Can you work these out from the model? Positions are in its coordinate system, mm. Give positions to 0.01 mm unless a question says otherwise; leave off trailing zeros. Loops run counter-clockwise (first coordinate to the right, second up) from the corner with the lowest first, then second, coordinate; pieces in that order, holes last. Notation, with made-up numbers: (-37.75, -18) - (-25.75, -18) arc R23 ccw to (-25.75, 18) - close; hole circle Ø3 at (-8, -30). An arc over 180 degrees is marked (long way). Write item = value, one per line.
from build123d import *

# Parameters (mm, degrees)
SKETCH_1_W          = 850
SKETCH_1_H          = 200
EXTRUDE_1_DEPTH     = 14
CUT_EXTRUDE_1_REACH = 438.831
SKETCH_2_W          = 235
SKETCH_2_H          = 70
FILLET_1_R          = 20


with BuildPart() as part:
    # 草图1 → 凸台-拉伸1 (new body)
    with BuildSketch(Plane.XY):
        Rectangle(SKETCH_1_W, SKETCH_1_H)
    extrude(amount=EXTRUDE_1_DEPTH)

    # 草图2 → 切除-拉伸1 (cut, up to next)
    with BuildSketch(Plane(origin=(0, 0, 0), x_dir=(-1, 0, 0), z_dir=(0, 0, -1)), mode=Mode.PRIVATE) as cut_extrude_1_sk1:
        with Locations((252.5, 65)):
            Rectangle(SKETCH_2_W, SKETCH_2_H)
    cut_extrude_1_tool1 = extrude(cut_extrude_1_sk1.sketch, amount=-CUT_EXTRUDE_1_REACH, mode=Mode.PRIVATE) & part.part
    # 草图2 → 切除-拉伸1 (cut, up to next)
    with BuildSketch(Plane(origin=(0, 0, 0), x_dir=(-1, 0, 0), z_dir=(0, 0, -1)), mode=Mode.PRIVATE) as cut_extrude_1_sk2:
        with Locations((-252.5, 65)):
            Rectangle(SKETCH_2_W, SKETCH_2_H)
    cut_extrude_1_tool2 = extrude(cut_extrude_1_sk2.sketch, amount=-CUT_EXTRUDE_1_REACH, mode=Mode.PRIVATE) & part.part
    add(cut_extrude_1_tool1.solids().sort_by_distance((-252.5, 65, 0))[0], mode=Mode.SUBTRACT)
    add(cut_extrude_1_tool2.solids().sort_by_distance((252.5, 65, 0))[0], mode=Mode.SUBTRACT)

    # 圆角1
    fillet_1_edges = [part.edges().sort_by_distance(p)[0] for p in [
        (-370, 30, 7),
        (-135, 30, 7),
        (135, 30, 7),
        (370, 30, 7),
    ]]
    fillet(fillet_1_edges, radius=FILLET_1_R)


solid = part.part
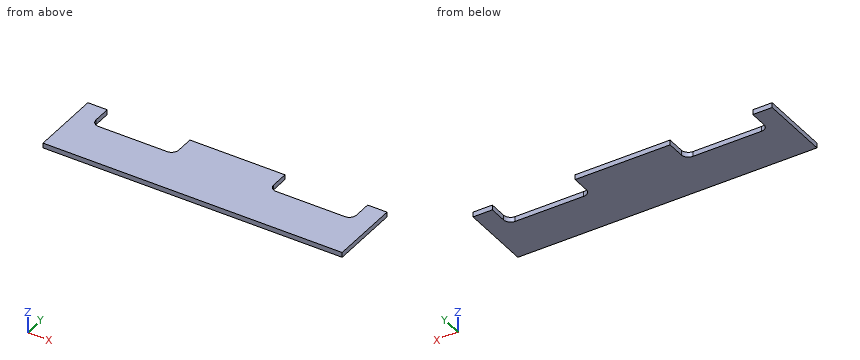
Q1. I need wall thicknesses on L1, parallel to X at y = 66, z = 7; L2, parallel to X at y = 44, z = 7; L3, parallel to Y at x = -257, z = 8.75. Which ranges of each line are inside material? Lowest first, please.
Output:
L1 = -425 to -370, -135 to 135, 370 to 425
L2 = -425 to -369.08, -135.92 to 135.92, 369.08 to 425
L3 = -100 to 30
Q2. Imagine slicing it at A-A, the plane z = 7.5. Write out the boundary of the cut face in (x, y).
Output:
outline = (-425, -100) - (425, -100) - (425, 100) - (370, 100) - (370, 50) arc R20 cw to (350, 30) - (155, 30) arc R20 cw to (135, 50) - (135, 100) - (-135, 100) - (-135, 50) arc R20 cw to (-155, 30) - (-350, 30) arc R20 cw to (-370, 50) - (-370, 100) - (-425, 100) - close
Q3. Imagine slicing it at B-B, the plane y = 41. Write out the boundary of the cut face in (x, z).
Output:
outline = (-425, 0) - (-367.86, 0) - (-367.86, 14) - (-425, 14) - close; (-137.14, 0) - (137.14, 0) - (137.14, 14) - (-137.14, 14) - close; (367.86, 0) - (425, 0) - (425, 14) - (367.86, 14) - close
Q4. Imagine slicing it at C-C, the plane x = -275. Write out the boundary of the cut face in (y, z).
Output:
outline = (-100, 0) - (30, 0) - (30, 14) - (-100, 14) - close
Q5. For pin 1 (7 mm diameter, centred on x = -282, z = 4, fed in from +Y), with a flat end and sliding along its axis, tell me the tip position at first contact or that it passes through.
Output:
pin_1 = 30
